```python
from build123d import *

# Parameters (mm, degrees)
BOSS_EXTRUDE1_DEPTH = 32
CHAMFER1_SIZE       = 5
SKETCH2_R           = 10.75
BOSS_EXTRUDE2_DEPTH = 3
HOLE2_D             = 5.5
HOLE2_DEPTH         = 100
HOLE2_CBORE_D       = 10
HOLE2_CBORE_DEPTH   = 7
CHAMFER3_SIZE       = 3
HOLE3_D             = 17
CHAMFER5_SIZE       = 0.5
CHAMFER6_SIZE       = 1


with BuildPart() as part:
    # Sketch1 → Boss-Extrude1 (new body)
    with BuildSketch(Plane.XY):
        Polygon((11.5, -16.008629624), (-11.5, -16.008629624), (-11.5, -0.008629624), (-27, -0.008629624), (-27, 9.991370376), (27, 9.991370376), (27, -0.008629624), (11.5, -0.008629624), align=None)
    extrude(amount=BOSS_EXTRUDE1_DEPTH)

    # Chamfer1
    chamfer1_edges = [part.edges().sort_by_distance(p)[0] for p in [
        (-27, 4.991370376, 0),
        (27, 4.991370376, 0),
        (-27, 4.991370376, 32),
        (27, 4.991370376, 32),
    ]]
    chamfer(chamfer1_edges, length=CHAMFER1_SIZE)

    # Sketch2 → Boss-Extrude2 (add)
    with BuildSketch(Plane(origin=(0, 9.991370376, 0), x_dir=(1, 0, 0), z_dir=(0, 1, 0))):
        with Locations(Location((0, -16.547126345, 0), (0, 0, 270))):
            Circle(SKETCH2_R)
    extrude(amount=BOSS_EXTRUDE2_DEPTH)

    # Hole2
    with Locations(Plane(origin=(0, -0.008629624, 0), x_dir=(-1, 0, 0), z_dir=(0, -1, 0))):
        with Locations((-20, -16), (20, -16)):
            CounterBoreHole(HOLE2_D / 2, HOLE2_CBORE_D / 2, HOLE2_CBORE_DEPTH, depth=HOLE2_DEPTH)

    # Chamfer3
    chamfer3_edges = [part.edges().sort_by_distance(p)[0] for p in [
        (-11.5, -8.008629624, 32),
        (11.5, -8.008629624, 32),
        (11.5, -8.008629624, 0),
        (-11.5, -8.008629624, 0),
    ]]
    chamfer(chamfer3_edges, length=CHAMFER3_SIZE)

    # Hole3 (through all)
    with Locations(Plane(origin=(0, -16.008629624, 0), x_dir=(-1, 0, 0), z_dir=(0, -1, 0))):
        with Locations((0, -16)):
            Hole(HOLE3_D / 2)

    # Chamfer5
    chamfer5_edges = [part.edges().sort_by_distance(p)[0] for p in [
        (-8.5, 12.991370376, 16),
    ]]
    chamfer(chamfer5_edges, length=CHAMFER5_SIZE)

    # Chamfer6
    chamfer6_edges = [part.edges().sort_by_distance(p)[0] for p in [
        (-8.5, -16.008629624, 16),
    ]]
    chamfer(chamfer6_edges, length=CHAMFER6_SIZE)


solid = part.part
```
The listing builds one solid part. Answer for the finished solid, in the listing's coordinates (mm). A direction names the side the tool comes from. Round coordinates to 2 decimals unless told otherwise and drop trailing zeros. Loops run counter-clockwise (first coordinate to the right, second up) from the corner with the lowest first, then second, coordinate; pieces in that order, holes last.
1) A cutting plane is placed at C-C on z = 30. Determine the outline of the cut face in (x, y), plus the area to 3 significant figures.
Outcome:
outline: (-24, -0.01) - (-10.5, -0.01) - (-10.5, -16.01) - (10.5, -16.01) - (10.5, -0.01) - (24, -0.01) - (24, 9.99) - (-24, 9.99) - close
area: 816 mm2
2) For faces 4 (the face through (17.8, 6.991, 18.2)), 5 (the face through (-10, -8.1, 1.5)), 6 (the face through (11.5, -8, 16)), determine the directions among +Z, -Z, +X, -X, +Y, -Y from which every point of the face is accessible in a straight line to the end or side of a thin tool.
Outcome:
face 4: -Y
face 5: -Z, -X, -Y
face 6: +Z, -Z, +X, -Y
3) A cutting plane is placed at A-A on x = 0. Determine the outline of the cut face in (y, z).
Outcome:
outline: (-16.01, 0) - (9.99, 0) - (9.99, 5.8) - (12.99, 5.8) - (12.99, 7) - (12.49, 7.5) - (-15.01, 7.5) - (-16.01, 6.5) - close; (-16.01, 25.5) - (-15.01, 24.5) - (12.49, 24.5) - (12.99, 25) - (12.99, 27.3) - (9.99, 27.3) - (9.99, 32) - (-16.01, 32) - close
4) A cutting plane is placed at B-B on y = -4. Determine the outline of the cut face in (x, z), plus the area to 3 significant figures.
Outcome:
outline: (-11.5, 3) - (-8.5, 0) - (8.5, 0) - (11.5, 3) - (11.5, 29) - (8.5, 32) - (-8.5, 32) - (-11.5, 29) - close; hole circle Ø17 at (0, 16)
area: 491 mm2
5) For a pull along X with two mould halves and no side action, classify faces 1 (the face through (-1.84, -1.07, 24.3)), 2 (the face through (3.23, 11.47, 26.8)), 3 (the face through (0, 9.991, 5)) as released by +X, released by -X, zero draft, split by the parting line, or undercut.
Outcome:
face 1: undercut
face 2: split by the parting line
face 3: zero draft
6) A cutting plane is placed at D-D on y = 4.75. Determine the outline of the cut face in (x, z), plus the area to 3 significant figures.
Outcome:
outline: (-27, 5) - (-22, 0) - (22, 0) - (27, 5) - (27, 27) - (22, 32) - (-22, 32) - (-27, 27) - close; hole circle Ø10 at (-20, 16); hole circle Ø17 at (0, 16); hole circle Ø10 at (20, 16)
area: 1,290 mm2
7) Consider line 1 (X direction, y = 9.3, z = 16); line 2 (X direction, y = 3.5, z = 16); line 3 (Z direction, x = 20, y = 2). Determine where each line is inside the solid, lowest interval first.
Outcome:
line 1: x = -27 to -22.75, -17.25 to -8.5, 8.5 to 17.25, 22.75 to 27
line 2: x = -27 to -25, -15 to -8.5, 8.5 to 15, 25 to 27
line 3: z = 0 to 11, 21 to 32
8) Given P1, Ø8, axis at x = 20.5, z = 15, coming from the -Y side; P2, Ø10, axis at y = -4.5, z = 12.5, coming from the -X side; P3, Ø5, axis at x = 20, z = 16, coming from the +Y side; P4, Ø8, axis at x = 20, z = 16, coming from the +Y side, each flat-ended and moving along its own axis, determine where each tip first touches the part or whether it passes through.
Outcome:
P1: stops at y = -0.01
P2: stops at x = -27
P3: passes through
P4: stops at y = 9.99
